from build123d import *

# Parameters (mm, degrees)
EXTRUDE_1_DEPTH        = 8
PATTERN_LINEAR_1_COUNT = 10
PATTERN_LINEAR_1_PITCH = 55
PATTERN_LINEAR_2_COUNT = 8
PATTERN_LINEAR_2_PITCH = 50
SKETCH_6_R             = 30
CUT_EXTRUDE_1_DEPTH    = 672.551189411


with BuildPart() as part:
    # 草图1 → 凸台-拉伸1 (new, symmetric)
    with BuildSketch(Plane.XY):
        Polygon((0, 0), (385, 0), (385, 50), (50, 550), (0, 550), align=None)
    extrude(amount=EXTRUDE_1_DEPTH, both=True)

    # 草图3 → M8 螺纹孔1 (revolve, cut)
    with BuildSketch(Plane.ZX.offset(520)):
        Polygon((0, 0), (0, 24.292926105), (3.4, 22.25), (3.4, 0), align=None)
    hole_wizard_m8_1 = revolve(axis=Axis((-6.35, 520, 0), (1, 0, 0)), mode=Mode.SUBTRACT)

    # 阵列(线性)1: M8 螺纹孔1 ×10
    with Locations(*[(0, -i * PATTERN_LINEAR_1_PITCH, 0) for i in range(1, PATTERN_LINEAR_1_COUNT)]):
        add(hole_wizard_m8_1, mode=Mode.SUBTRACT)

    # 草图5 → M8 螺纹孔2 (revolve, cut)
    with BuildSketch(Plane(origin=(20, 0, 0), x_dir=(0, 0, -1), z_dir=(1, 0, 0))):
        Polygon((0, 0), (0, 24.292926105), (3.4, 22.25), (3.4, 0), align=None)
    hole_wizard_m8_2 = revolve(axis=Axis((20, -6.35, 0), (0, 1, 0)), mode=Mode.SUBTRACT)

    # 阵列(线性)2: M8 螺纹孔2 ×8
    with Locations(*[(i * PATTERN_LINEAR_2_PITCH, 0, 0) for i in range(1, PATTERN_LINEAR_2_COUNT)]):
        add(hole_wizard_m8_2, mode=Mode.SUBTRACT)

    # 草图6 → 切除-拉伸1 (cut, through all)
    with BuildSketch(Plane(origin=(0, 0, -8), x_dir=(-1, 0, 0), z_dir=(0, 0, -1))):
        with Locations((-285, 70)):
            Circle(SKETCH_6_R)
        with Locations((-129.147552133, 302.615593832)):
            Circle(SKETCH_6_R)
        with Locations((-207.073776066, 186.307796916)):
            Circle(SKETCH_6_R)
        with Locations((-135, 70)):
            Circle(SKETCH_6_R)
        with Locations((-51.221328199, 418.923390748)):
            Circle(SKETCH_6_R)
        with Locations((-57.073776066, 186.307796916)):
            Circle(SKETCH_6_R)
    extrude(amount=-CUT_EXTRUDE_1_DEPTH, mode=Mode.SUBTRACT)


solid = part.part
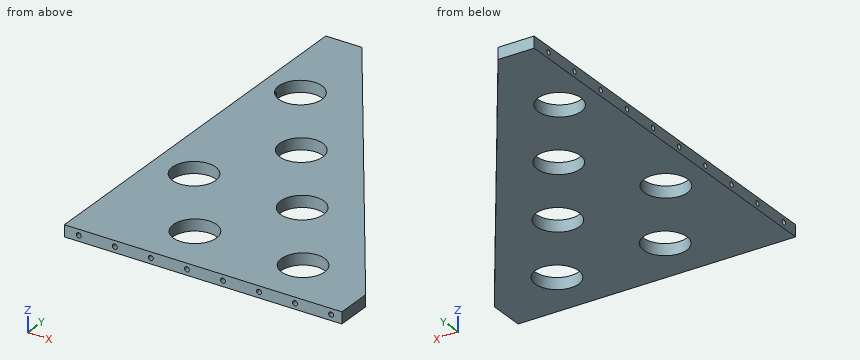
Source: CAD feature listing. Evaluate the final solid. Frame: model axes, mm. Round coordinates to 2 decimals unless told otherwise and drop trailing zeros. Loops run counter-clockwise (first coordinate to the right, second up) from the corner with the lowest first, then second, coordinate; pieces in that order, holes last. Notation, with made-up numbers: (-12.75, 58.25) -> (35.25, 58.25) arc R14 ccw to (35.25, 68.25) -> close; hole circle Ø10 at (75.25, -14). An arc over 180 degrees is marked (long way). Answer as a JSON object with one key per item and string values. Group by question number.
Q1. Ray query, line 1 (Z direction, x = 220, y = 14.5); line 2 (Y direction, x = 135, z = 3); line 3 (X direction, y = 177.5, z = -4.5) (3 decimals). Return the intervals inside material, ascending. Write a range as from..to.
Q2. Section query C-C (x = 280). Output: boundary loops of the cut face in (y, z), plus the area to 3 significant figures.
Q3. Contact query for flat-ended pins moving along their axis: P1, Ø5.5, axis at y = 520, z = 0, coming from the +X side; P2, Ø6, axis at y = 135, z = 0, coming from the -X side; P3, Ø5.5, axis at x = 220, z = 0, coming from the +Y side. Output: stop coordinate, or through.
Q4. Section query B-B (y = 62). Output: boundary loops of the cut face in (x, z).
Q5. Section query A-A (x = 143). Output: boundary loops of the cut face in (y, z), plus the area to 3 significant figures.
Completed:
{
 "1": {"line 1": "-8..-3.4, 3.4..8", "line 2": "0..40, 100..273.19, 332.04..423.13", "line 3": "0..28.396, 85.752..178.396, 235.752..299.575"},
 "2": {"outline": "(0, -8) -> (40.42, -8) -> (40.42, 8) -> (0, 8) -> close; (99.58, -8) -> (206.72, -8) -> (206.72, 8) -> (99.58, 8) -> close", "area": "2,360 mm²"},
 "3": {"P1": "x = 71.94", "P2": "x = 22.49", "P3": "y = 300.37"},
 "4": {"outline": "(0, -8) -> (106.09, -8) -> (106.09, 8) -> (0, 8) -> close; (163.91, -8) -> (256.09, -8) -> (256.09, 8) -> (163.91, 8) -> close; (313.91, -8) -> (376.96, -8) -> (376.96, 8) -> (313.91, 8) -> close"},
 "5": {"outline": "(0, -8) -> (41.09, -8) -> (41.09, 8) -> (0, 8) -> close; (98.91, -8) -> (276.01, -8) -> (276.01, 8) -> (98.91, 8) -> close; (329.23, -8) -> (411.19, -8) -> (411.19, 8) -> (329.23, 8) -> close", "area": "4,800 mm²"}
}
